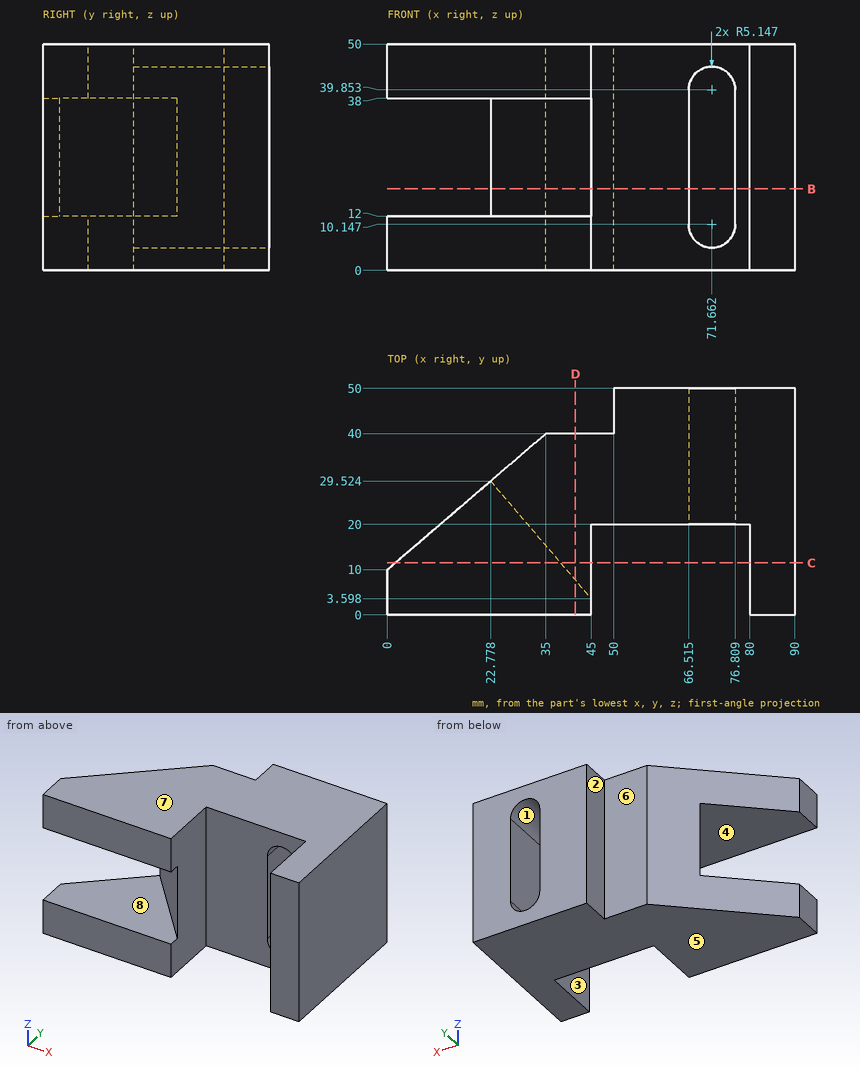
Geometry check sheet. Reference: drawing and pictorial views, mm from the part's lowest x, y, z. A direction names the side the tool comes from. Give positions to 0.01 mm unless a question says otherwise; leave off trailing zeros. Order: outer loops, then holes, each group sorted by start corner. A loop starts at its lowest first (then second) coordinate and runs counter-clockwise, first axis right, second up. Notation, with made-up numbers: (47.5, -31) - (87.5, -31) arc R21 cw to (87.5, -21) - close; hole circle Ø8 at (46, 38.25). An arc over 180 degrees is marked (long way). Answer as CSV lines item,"result".
1. Section check B-B (z = 18). Record the boundary of the cut face in (x, y) (1 decimal).
Result sheet:
outline,"(22.8, 29.5) - (45, 3.6) - (45, 20) - (66.5, 20) - (66.5, 50) - (50, 50) - (50, 40) - (35, 40) - close; (76.8, 20) - (80, 20) - (80, 0) - (90, 0) - (90, 50) - (76.8, 50) - close"
2. Section check C-C (y = 11.5). Record the boundary of the cut face in (x, z), then the cut area to 3 significant figures.
Result sheet:
outline,"(1.75, 0) - (45, 0) - (45, 50) - (1.75, 50) - (1.75, 38) - (38.23, 38) - (38.23, 12) - (1.75, 12) - close; (80, 0) - (90, 0) - (90, 50) - (80, 50) - close"
area,"1,710 mm²"
3. Mould release check, pull along Z, two halves, no side actions. Record for the marked faces 5, 6, 7 and 8: released by +Z, released by -Z, zero draft, split by the parting line, or undercut.
Result sheet:
face 5,"released by -Z"
face 6,"zero draft"
face 7,"released by +Z"
face 8,"undercut"
4. Go/stop test with flat-tipped pins: P1, Ø5, axis at y = 45, z = 32.5, coming from the -X side; P2, Ø10, axis at x = 50.5, y = 5.5, coming from the +Z side; P3, Ø3, axis at x = 77, z = 14, coming from the -Y side; P4, Ø16, axis at y = 6.5, z = 23, coming from the -X side (1 decimal). Record where each tip stops, or that it passes through.
Result sheet:
P1,"x = 50"
P2,"through"
P3,"y = 20"
P4,"x = 35.7"
5. Tool access check on the marked faces 1, 2, 3 and 4. Record the directions out of +Z, -Z, +X, -X, +Y, -Y that give a thin tool (end or side, any length) a straight path to the whole face; none if there is none.
Result sheet:
face 1,"+Y, -Y"
face 2,"+Z, -Z, -X, +Y"
face 3,"+Z, -Z, -Y"
face 4,"-X, -Y"
6. Scan lines: probe 1 along Z at (x, y) = (6, 12); probe 2 along X at (y, z) = (5, 40.5); probe 3 along X at (y, z) = (43, 22) (1 decimal). Record each from-to range of solid material in increasing order. Write a range as from..to.
Result sheet:
probe 1,"0..12, 38..50"
probe 2,"0..45, 80..90"
probe 3,"50..66.5, 76.8..90"
7. Section check D-D (x = 41.5). Record the boundary of the cut face in (y, z), then the cut area to 3 significant figures.
Result sheet:
outline,"(0, 0) - (40, 0) - (40, 50) - (0, 50) - (0, 38) - (7.68, 38) - (7.68, 12) - (0, 12) - close"
area,"1,800 mm²"
